Print and shaded views of the part. All mm, measured from the part's lowest x, y and z. Round coordinates to 2 decimals unless told otherwise and drop trailing zeros. Loops run counter-clockwise (first coordinate to the right, second up) from the corner with the lowest first, then second, coordinate; pieces in that order, holes last. Notation, with made-up numbers: (89, 71) -> (121, 71) arc R22 cw to (121, 86) -> close; hole circle Ø10 at (-35, -38). An arc over 180 degrees is marked (long way). Use a Markdown table: item, result.
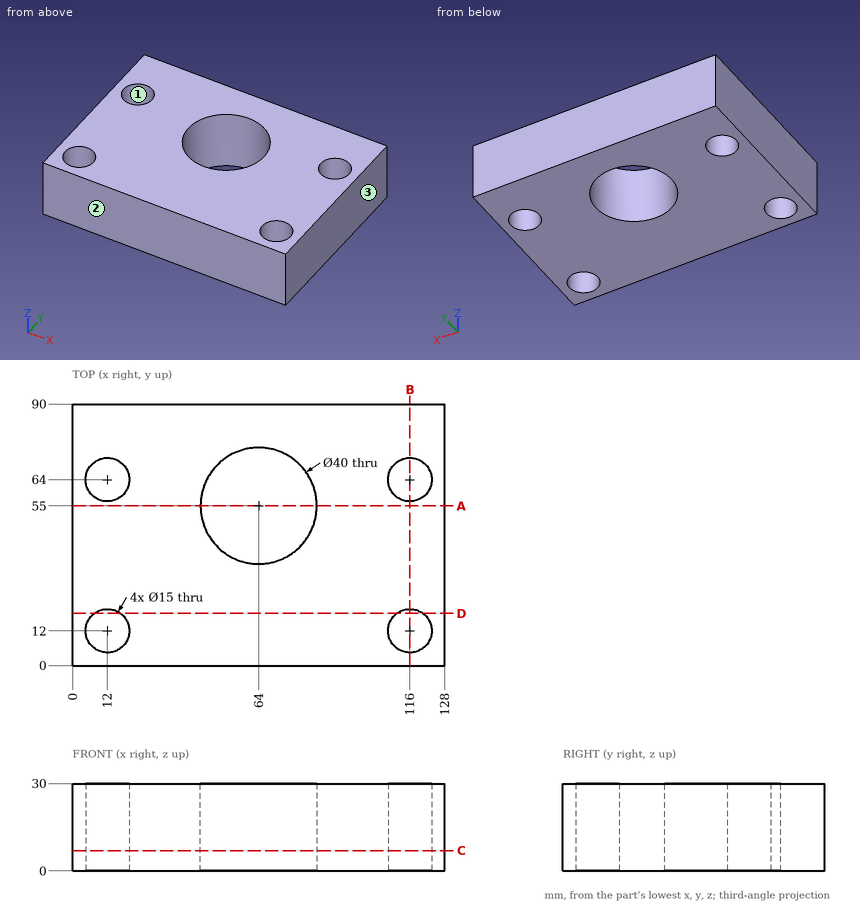
Q1. Band-saw the part on D-D, the plane y = 18. Give the cut face in (x, z).
Results list:
| item | result |
|---|---|
| outline | (0, 0) -> (7.5, 0) -> (7.5, 30) -> (0, 30) -> close; (16.5, 0) -> (111.5, 0) -> (111.5, 30) -> (16.5, 30) -> close; (120.5, 0) -> (128, 0) -> (128, 30) -> (120.5, 30) -> close |
Q2. Band-saw the part on C-C, the plane z = 7. Give the cut face in (x, y), plus the area to 3 significant figures.
Results list:
| item | result |
|---|---|
| outline | (0, 0) -> (128, 0) -> (128, 90) -> (0, 90) -> close; hole circle Ø15 at (12, 12); hole circle Ø15 at (12, 64); hole circle Ø40 at (64, 55); hole circle Ø15 at (116, 12); hole circle Ø15 at (116, 64) |
| area | 9,560 mm² |
Q3. Band-saw the part on A-A, the plane y = 55. Give the cut face in (x, z).
Results list:
| item | result |
|---|---|
| outline | (0, 0) -> (44, 0) -> (44, 30) -> (0, 30) -> close; (84, 0) -> (128, 0) -> (128, 30) -> (84, 30) -> close |
Q4. Flat gauge pin, fed straight in: pin 1 (12 mm diameter, centred on x = 12, y = 64, fed in from +Z). Where does the tip first touch, or does it go through?
Results list:
| item | result |
|---|---|
| pin 1 | passes through |
Q5. Pull direction Y, two halves, no side cores. Call the marked faces 1, 2 and 3: released by +Y, released by -Y, zero draft, split by the parting line, or undercut.
Results list:
| item | result |
|---|---|
| face 1 | undercut |
| face 2 | released by -Y |
| face 3 | zero draft |
Q6. Band-saw the part on B-B, the plane x = 116. Give the cut face in (y, z), plus the area to 3 significant figures.
Results list:
| item | result |
|---|---|
| outline | (0, 0) -> (4.5, 0) -> (4.5, 30) -> (0, 30) -> close; (19.5, 0) -> (56.5, 0) -> (56.5, 30) -> (19.5, 30) -> close; (71.5, 0) -> (90, 0) -> (90, 30) -> (71.5, 30) -> close |
| area | 1,800 mm² |
Q7. Drill centre lines: L1, parallel to Y at x = 116, z = 17; L2, parallel to Y at x = 64, z = 17.5; L3, parallel to X at y = 7.5, z = 27. Where is each one in solid material? Low to high. Write a range as from..to.
Results list:
| item | result |
|---|---|
| L1 | y = 0..4.5, 19.5..56.5, 71.5..90 |
| L2 | y = 0..35, 75..90 |
| L3 | x = 0..6, 18..110, 122..128 |
